from build123d import *

# Parameters (mm, degrees)
SKETCH1_R               = 3
BOSS_EXTRUDE1_DEPTH     = 8
CUT_EXTRUDE1_DEPTH      = 10
CUT_EXTRUDE1_DEPTH_BACK = 10
SKETCH2_W               = 30
SKETCH2_H               = 6
BOSS_EXTRUDE2_DEPTH     = 5
SCALE1_SCALE            = 0.5


with BuildPart() as part:
    # Sketch1 → Boss-Extrude1 (new body)
    with BuildSketch(Plane.XY):
        with BuildLine():
            Line((-59.466854234, -95.453658304), (-34.265346163, -6.824512068))
            ThreePointArc((-34.265346163, -6.824512068), (-30.086435736, -0.093123284), (-22.875098798, -3.375120677))
            ThreePointArc((-22.875098798, -3.375120677), (-18.350652777, -6.324611935), (-13.784422872, -3.44023073))
            ThreePointArc((-13.784422872, -3.44023073), (-5.593314668, -0.648514381), (-3.132391837, -8.945007172))
            ThreePointArc((-3.132391837, -8.945007172), (-3.598758132, -10.251856882), (-3.590598772, -11.639404038))
            Line((-3.590598772, -11.639404038), (-4.345412305, -7.496284288))
            Line((-4.345412305, -7.496284288), (-48.279353466, -99.676151096))
            ThreePointArc((-48.279353466, -99.676151096), (-55.814324496, -102.708171614), (-59.466854234, -95.453658304))
        make_face()
        with Locations((-28.347406658, -5.835577277)):
            Circle(SKETCH1_R, mode=Mode.SUBTRACT)
        with Locations((-8.347919622, -5.978819396)):
            Circle(SKETCH1_R, mode=Mode.SUBTRACT)
    extrude(amount=BOSS_EXTRUDE1_DEPTH)

    # Sketch2 → Cut-Extrude1 (cut, two sides: drawn at the far end of the back side and taken through both)
    with BuildSketch(Plane(origin=(0, 0, 0), x_dir=(1, 0, 0), z_dir=(0, 1, 0)).offset(-CUT_EXTRUDE1_DEPTH_BACK)):
        with Locations((-2.347919622, -4)):
            Rectangle(SKETCH2_W, SKETCH2_H)
    extrude(amount=CUT_EXTRUDE1_DEPTH + CUT_EXTRUDE1_DEPTH_BACK, mode=Mode.SUBTRACT)

    # Sketch3 → Boss-Extrude2 (add)
    with BuildSketch(Plane.XY.offset(8)):
        with BuildLine():
            Line((-16.158374435, -32.281615332), (-41.189011455, -31.173790769))
            Line((-41.189011455, -31.173790769), (-59.466854234, -95.453658304))
            ThreePointArc((-59.466854234, -95.453658304), (-55.814324496, -102.708171614), (-48.279353466, -99.676151096))
            Line((-48.279353466, -99.676151096), (-16.158374435, -32.281615332))
        make_face()
    boss_extrude2 = extrude(amount=BOSS_EXTRUDE2_DEPTH)

    # Mirror1: Boss-Extrude2 across plane
    add(boss_extrude2.mirror(Plane.XY.offset(4)))


with BuildPart() as part_1:
    # Scale1: scaled about (0, 0, 0)
    add(part.part.scale(SCALE1_SCALE))


solid = part_1.part
Input: part model. Units: mm. Frame: model coordinates. A direction names the side the tool comes from. Give positions to 0.01 mm unless a question says otherwise; leave off trailing zeros. Order: outer loops, then holes, each group sorted by start corner. A loop starts at its lowest first (then second) coordinate and runs counter-clockwise, first axis right, second up. Notation, with made-up numbers: (-12.5, -5.75) - (39.5, -5.75) arc R21 ccw to (39.5, 24.25) - close; hole circle Ø11 at (34, -16). An arc over 180 degrees is marked (long way). Answer as a JSON object with one key per item and string values. Group by question number.
Q1. Mould query, pull axis Z, two halves, no side actions, for faces 4 (the face through (-6, -5, 2)), 5 (the face through (-2.857, -0.294, 3.746)), 6 (the face through (-19, -33, 6.5)), 7 (the face through (-8.674, -4, 2)). Classes: pulls with the +Z half, pulls with the -Z half, needs draft (parallel to the pull), parting line crosses it, or undercut.
Q2. Cut plane B-B, the plane x = -4.75. Output: boundary loops of the cut face in (y, z).
Q3. Cut plane C-C, the plane y = -29. Output: boundary loops of the cut face in (x, z).
Q4. Cut plane D-D, the plane x = -14. Output: boundary loops of the cut face in (y, z).
Q5. Set-up query: faces 1 (the face through (-19, -33, -2.5)), 2 (the face through (-6, -3, 3.5)), 3 (the face through (-14.249, -15.868, 5.232)). Return all of +Z, -Z, +X, -X, +Y, -Y with unobstructed straight access to the full face (end or side cutting, diameter ignored); none if empty.
Q6. Cut plane A-A, the plane z = 2.75. Output: boundary loops of the cut face in (x, y), then the cut area to 3 significant figures.
Q7. First-contact query: pin 1 Ø1.8 at (x, y) = (-14.17, -2.92) entering from -Z; pin 2 Ø13 at (x, y) = (-11.5, -9) entering from +Z; pin 3 Ø4 at (x, z) = (-22.5, 3.5) entering from -Y; pin 4 Ø2 at (y, z) = (-10, 3.5) entering from -X. Flat tips, straight axial feed; report the tip coordinate or a pass-through.
Q8. Line query: probe 1 along Z at (x, y) = (-5.5, -10); probe 2 along X at (y, z) = (-3.5, 3.75); probe 3 along X at (y, z) = (-23.5, 4). Output: solid intervals per line, ascending.
Results:
{
 "1": {"face 4": "undercut", "face 5": "needs draft", "face 6": "pulls with the +Z half", "face 7": "undercut"},
 "2": {"outline": "(-9.16, 0) - (-4.37, 0) - (-4.37, 0.5) - (-5, 0.5) - (-5, 3.5) - (-4.37, 3.5) - (-4.37, 4) - (-9.16, 4) - close; (-1.6, 0) - (-0.05, 0) - (-0.05, 0.5) - (-1.6, 0.5) - close; (-1.6, 3.5) - (-0.05, 3.5) - (-0.05, 4) - (-1.6, 4) - close"},
 "3": {"outline": "(-24.41, -2.5) - (-14.21, -2.5) - (-14.21, 6.5) - (-24.41, 6.5) - close"},
 "4": {"outline": "(-28.56, -2.5) - (-15.88, -2.5) - (-15.88, 0) - (-4.41, 0) - (-4.41, 4) - (-15.88, 4) - (-15.88, 6.5) - (-28.56, 6.5) - close; (-1.43, 0) - (0.08, 0) - (0.08, 4) - (-1.43, 4) - close"},
 "5": {"face 1": "-Z, +X, -X, +Y, -Y", "face 2": "+X, +Y", "face 3": "+Z, +X, +Y"},
 "6": {"outline": "(-29.73, -47.73) arc R3 ccw to (-24.14, -49.84) - (-2.77, -5) - (-8.67, -5) - (-8.67, -3.12) arc R2.5 cw to (-11.44, -1.69) arc R3 ccw to (-17.13, -3.41) - close; (-1.94, -5) - (-1.8, -5.82) arc R2 cw to (-1.77, -5) - close; hole circle Ø3 at (-14.17, -2.92)", "area": "502 mm^2"},
 "7": {"pin 1": "through", "pin 2": "z = 4", "pin 3": "y = -50.41", "pin 4": "x = -19.29"},
 "8": {"probe 1": "0 to 4", "probe 2": "-17.16 to -15.56, -12.79 to -5.58, -2.76 to -1.22", "probe 3": "-22.84 to -11.59"}
}
